Input: dimensioned drawing with shaded views. Units: mm. Origin: part minimum x, y, z. Coordinates: 2 decimals unless noted, no trailing zeros. Loops run counter-clockwise (first coordinate to the right, second up) from the corner with the lowest first, then second, coordinate; pieces in that order, holes last.
Item 1: Ray query, line 1 along Y through (x, z) = (10, 2); line 2 along X through (y, z) = (20, 2.75); line 3 along Y through (x, z) = (11, 9.75). Return the intervals inside material, ascending.
Item 2: Section B-B on x = 10. Return loops of the section in (y, z), and give its area (3 significant figures).
Item 3: Section A-A on y = 20. Return loops of the section in (x, z), and give its area (3 significant figures).
Item 4: Contact query for a flat-ended pin moving along its axis: P1, Ø5.5, axis at x = 10, y = 380, coming from the -Z side. Output: stop coordinate, or through.
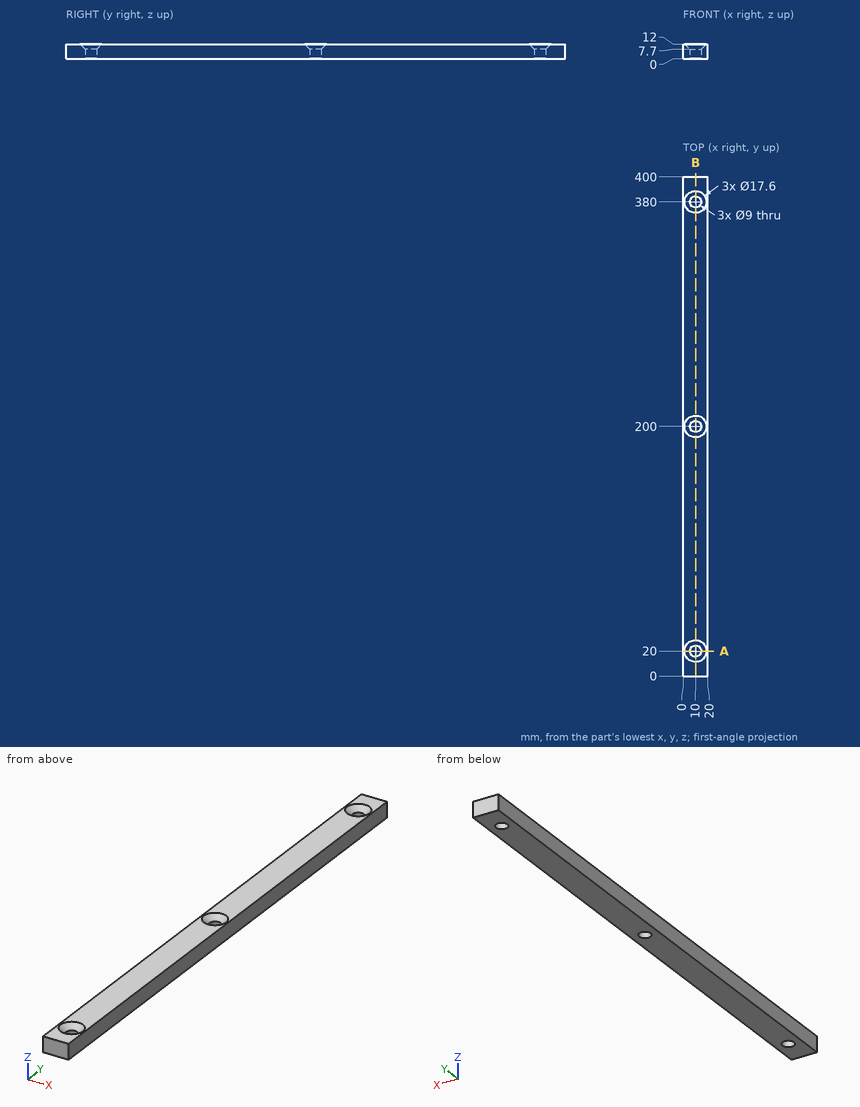
Results found:
1. line 1: y = 0 to 15.5, 24.5 to 195.5, 204.5 to 375.5, 384.5 to 400
1. line 2: x = 0 to 5.5, 14.5 to 20
1. line 3: y = 0 to 13.53, 26.47 to 193.53, 206.47 to 373.53, 386.47 to 400
2. outline: (0, 0) - (15.5, 0) - (15.5, 7.7) - (11.2, 12) - (0, 12) - close; (24.5, 0) - (195.5, 0) - (195.5, 7.7) - (191.2, 12) - (28.8, 12) - (24.5, 7.7) - close; (204.5, 0) - (375.5, 0) - (375.5, 7.7) - (371.2, 12) - (208.8, 12) - (204.5, 7.7) - close; (384.5, 0) - (400, 0) - (400, 12) - (388.8, 12) - (384.5, 7.7) - close
2. area: 4,420 mm2
3. outline: (0, 0) - (5.5, 0) - (5.5, 7.7) - (1.2, 12) - (0, 12) - close; (14.5, 0) - (20, 0) - (20, 12) - (18.8, 12) - (14.5, 7.7) - close
3. area: 114 mm2
4. P1: passes through
